Geometry check sheet. Reference: the model listing, model coordinates, mm. Face numbers are marked on the shaded views. Round coordinates to 2 decimals unless told otherwise and drop trailing zeros. Write each loop counter-clockwise with the first axis right and the second up, starting at its lowest first coordinate (ties: lowest second). Pieces come first, ordered by that corner, then holes. Notation, with made-up numbers: M 53.5,7.5 L 105.5,7.5 A34 ccw 105.5,40.5 Z; hole C 43,11 d1. An arc over 180 degrees is marked long. One line per item, written item: value. Start each with the question number.
1. Scan lines: probe 1 along X at (y, z) = (-50, 33); probe 2 along X at (y, z) = (-36, 15.5); probe 3 along Y at (x, z) = (77, 24). Record each from-to range of solid material in increasing order. Write a range as [from, to].
2. Section check B-B (z = 52). Record the boundary of the cut face in (x, y), and give its area (3 significant figures).
3. Depth check by flat-ended pin: P1, Ø5, axis at y = -9.5, z = 65.5, coming from the -X side; P2, Ø4, axis at x = 158.5, z = 31.5, coming from the -Y side; P3, Ø10, axis at x = 151, z = 39, coming from the -Y side. Enter the tip coordinate at first touch or a pass-through.
4. Section check C-C (y = -18.5). Record the boundary of the cut face in (x, z).
5. Section check A-A (y = -45). Record the boundary of the cut face in (x, z).
6. Release check for a two-part mould opening along X. For the marked faces 1, 2, 3 and 4 record: pulls with the +X half, pulls with the -X half, needs draft (parallel to the pull), parting line crosses it, or undercut.
7. Section check D-D (x = 38.5). Record the boundary of the cut face in (y, z) (3 decimals).
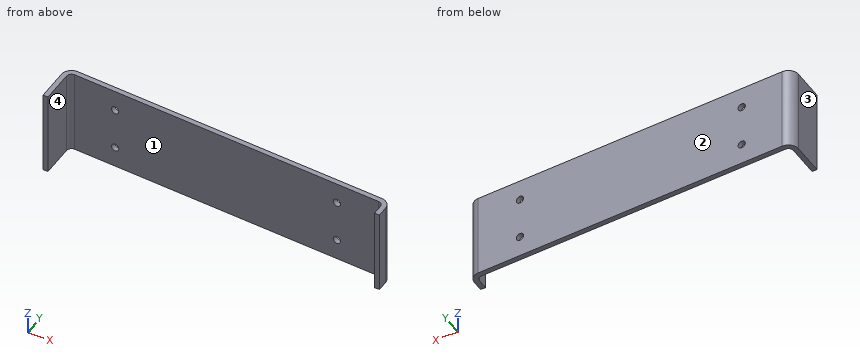
from build123d import *

# Parameters (mm, degrees)
BOSS_EXTRUDE1_DEPTH = 100
SKETCH4_R           = 4.5
CUT_EXTRUDE2_DEPTH  = 100
FILLET1_R           = 12
FILLET2_R           = 6


with BuildPart() as part:
    # Sketch1 → Boss-Extrude1 (new body)
    with BuildSketch(Plane.XY):
        Polygon((0, 0), (0, -52), (6, -52), (6, -6.434682036), (394, -33.594682036), (394, -52), (400, -52), (400, -28), align=None)
    extrude(amount=BOSS_EXTRUDE1_DEPTH)

    # Sketch4 → Cut-Extrude2 (cut)
    with BuildSketch(Plane(origin=(0, 0, 0), x_dir=(0.9975589671416267, -0.06982912769991385, 0), z_dir=(0.06982912769991385, 0.9975589671416267, 0))):
        with Locations(Location((63, -25, 0), (0, 0, 180))):
            Circle(SKETCH4_R)
        with Locations(Location((338, -25, 0), (0, 0, 180))):
            Circle(SKETCH4_R)
        with Locations(Location((63, -75, 0), (0, 0, 180))):
            Circle(SKETCH4_R)
        with Locations(Location((338, -75, 0), (0, 0, 180))):
            Circle(SKETCH4_R)
    extrude(amount=-CUT_EXTRUDE2_DEPTH, mode=Mode.SUBTRACT)

    # Fillet1
    fillet1_edges = [part.edges().sort_by_distance(p)[0] for p in [
        (400, -28, 50),
        (0, 0, 50),
    ]]
    fillet(fillet1_edges, radius=FILLET1_R)

    # Fillet2
    fillet2_edges = [part.edges().sort_by_distance(p)[0] for p in [
        (6, -6.434682036, 50),
        (394, -33.594682036, 50),
    ]]
    fillet(fillet2_edges, radius=FILLET2_R)


solid = part.part
Result sheet:
1. probe 1: x = [0, 6], [394, 400]
1. probe 2: x = [0, 6], [393.08, 399.57]
1. probe 3: y = [-11.4, -5.39]
2. outline: M 0,-52 L 6,-52 L 6,-12.87 A6 cw 12.42,-6.88 L 388.42,-33.2 A6 cw 394,-39.19 L 394,-52 L 400,-52 L 400,-39.19 A12 ccw 388.84,-27.22 L 12.84,-0.9 A12 ccw 0,-12.87 Z
2. area: 2,740 mm2
3. P1: stops at x = 0.03
3. P2: stops at y = -17.25
3. P3: stops at y = -16.93
4. outline: M 0,0 L 6,0 L 6,100 L 0,100 Z; M 178.36,0 L 264.29,0 L 264.29,100 L 178.36,100 Z
5. outline: M 0,0 L 6,0 L 6,100 L 0,100 Z; M 394,0 L 400,0 L 400,100 L 394,100 Z
6. face 1: undercut
6. face 2: pulls with the +X half
6. face 3: pulls with the -X half
6. face 4: undercut
7. outline: M -8.71,0 L -2.695,0 L -2.695,100 L -8.71,100 Z
